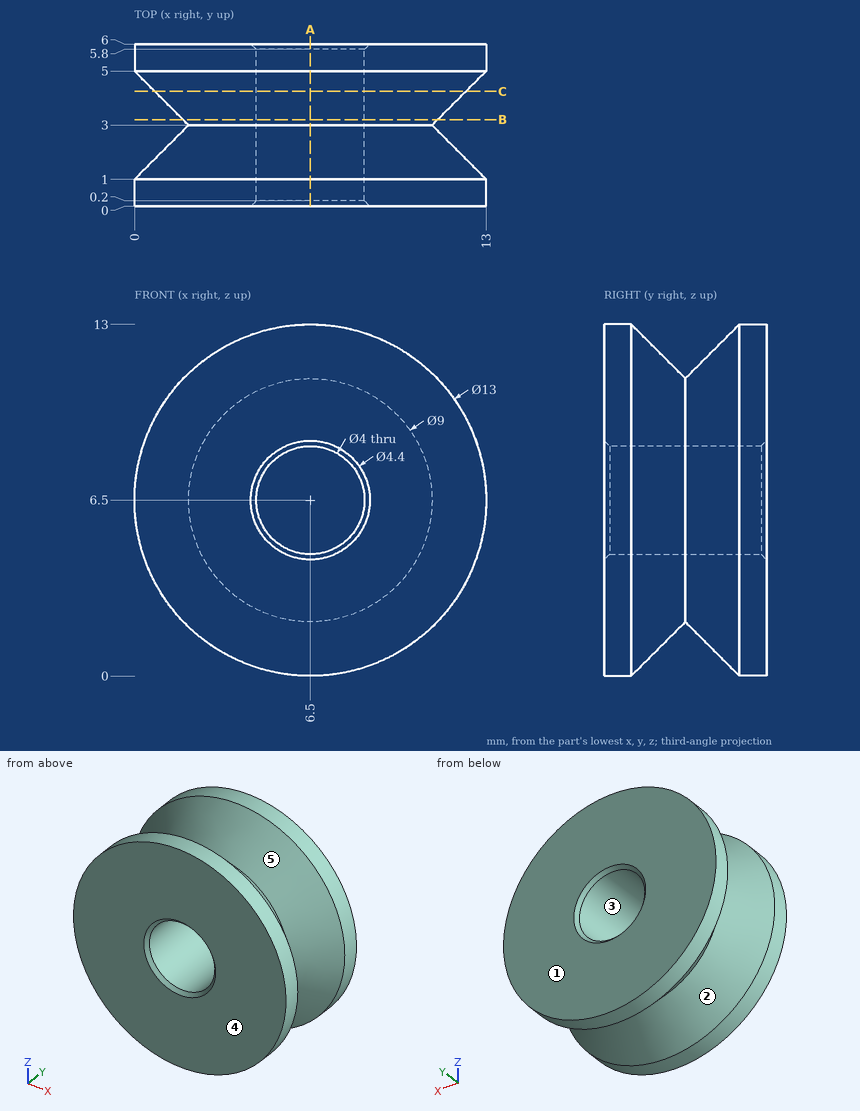
Source: three-view drawing plus pictorial views. Frame: mm from the lowest corner of the part. A direction names the side the tool comes from. Give positions to 0.01 mm unless a question says otherwise; leave off trailing zeros. Order: outer loops, then holes, each group sorted by start corner. A loop starts at its lowest first (then second) coordinate and runs counter-clockwise, first axis right, second up. Notation, with made-up numbers: (21.5, 6) - (55.5, 6) arc R17 ccw to (55.5, 23) - close; hole circle Ø6 at (21.5, 30). An arc over 180 degrees is marked (long way). Answer as a JSON object with one key per item and string values. Group by question number.
Q1. Cut plane A-A, the plane x = 6.5. Output: boundary loops of the cut face in (y, z), then the cut area to 3 significant figures.
Q2. Mould query, pull axis Z, two halves, no side actions, for the marked faces 1, 2 and 3. Classes: pulls with the +Z half, pulls with the -Z half, needs draft (parallel to the pull), parting line crosses it, or undercut.
Q3. Cut plane B-B, the plane y = 3.2. Output: boundary loops of the cut face in (x, z), then the cut area to 3 significant figures.
Q4. Set-up query: the marked faces 4 and 5. Return all of +Z, -Z, +X, -X, +Y, -Y with unobstructed straight access to the full face (end or side cutting, diameter ignored); none if empty.
Q5. Cut plane C-C, the plane y = 4.25. Output: boundary loops of the cut face in (x, z).
Q6. Line query: probe 1 along Y at (x, z) = (8.5, 1.5); probe 2 along X at (y, z) = (4.3, 6); probe 3 along X at (y, z) = (4.85, 1). Output: solid intervals per line, ascending.
Q7. First-contact query: pin 1 Ø3 at (x, z) = (9.5, 6.5) entering from -Y. Flat tip, straight axial feed; report the tip coordinate or a pass-through.
Results:
{
 "1": {"outline": "(0, 0) - (1, 0) - (3, 2) - (5, 0) - (6, 0) - (6, 4.3) - (5.8, 4.5) - (0.2, 4.5) - (0, 4.3) - close; (0, 8.7) - (0.2, 8.5) - (5.8, 8.5) - (6, 8.7) - (6, 13) - (5, 13) - (3, 11) - (1, 13) - (0, 13) - close", "area": "45.9 mm^2"},
 "2": {"face 1": "needs draft", "face 2": "parting line crosses it", "face 3": "undercut"},
 "3": {"outline": "circle Ø9.4 at (6.5, 6.5); hole circle Ø4 at (6.5, 6.5)", "area": "56.8 mm^2"},
 "4": {"face 4": "+Z, -Z, +X, -X, -Y", "face 5": "none"},
 "5": {"outline": "circle Ø11.5 at (6.5, 6.5); hole circle Ø4 at (6.5, 6.5)"},
 "6": {"probe 1": "0 to 2.11, 3.89 to 6", "probe 2": "0.72 to 4.56, 8.44 to 12.28", "probe 3": "3.33 to 9.67"},
 "7": {"pin 1": "y = 0"}
}
